Can you work these out from the model? Positions are in its coordinate system, mm. Face numbers are marked on the shaded views. A direction names the side the tool comes from. Coordinates: 2 decimals unless noted, no trailing zeros. Order: outer loops, then holes, each group sorted by start corner. A loop starts at its lowest first (then second) coordinate and runs counter-clockwise, first axis right, second up. Notation, with made-up numbers: M 59,65 L 95,65 A8 ccw 95,79 Z; hole C 33,-38 d2. An arc over 180 degrees is marked long. Answer as CSV lines item,"result". Start each with the question number.
1. I need wall thicknesses on line 1 along Z through (x, y) = (-30, 8.25); line 2 along Y through (x, z) = (-24, 19.5); line 3 along Y through (x, z) = (23, 33). Which ranges of each line are inside material? Lowest first, please. Write a range as from..to.
2. If we section it at A-A (x = 0): List the corners of the cut face in (y, z) for me, plus the area to 3 significant figures.
3. If we mould it in two halves opening along Y, with no side actions, what happens to the marked faces 6, 7 and 8? For each: released by +Y, released by -Y, zero draft, split by the parting line, or undercut.
4. Will these pins go through, and if not, where does the flat tip stop? pin 1 (3 mm diameter, centred on y = 23.5, z = 6.5, fed in from -X); pin 2 (3 mm diameter, centred on y = 25.5, z = 4.5, fed in from +X); pin 3 (2 mm diameter, centred on y = 45, z = 11.5, fed in from -X); pin 4 (8 mm diameter, centred on x = 36, z = 29, fed in from +Y).
5. If we section it at B-B (x = 31): List the corners of the cut face in (y, z) for me, plus the area to 3 significant figures.
6. On a 3-axis mill with a long thin cutter (end or side, diameter ignored), from which of +Z, -Z, +X, -X, +Y, -Y can I reach the whole of each face in a straight line? I mean the marked faces 1, 2, 3, 4 and 5. Say none if no direction works.
7. If we section it at C-C (z = 31.5): List the corners of the cut face in (x, y) for me.
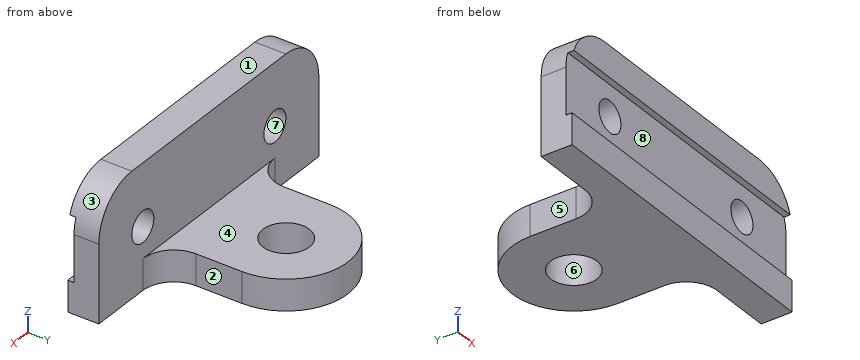
```python
from build123d import *
from OCP.BRepFilletAPI import BRepFilletAPI_MakeFillet

# Parameters (mm, degrees)
BASE_AND_EAR_PROFILE_SKETCH_W       = 100
BASE_AND_EAR_PROFILE_SKETCH_H       = 10
BASE_PLATE_DEPTH                    = 40
SKETCH1_3_R                         = 20
SKETCH1_3_R_2                       = 7.5
CLEVIS_EAR_DEPTH                    = 10
MOUNTING_HOLES_2X_REACH             = 80.262
MOUNTING_HOLES_SKETCH_R             = 5
MOUNTING_HOLES_2X_DIRECTION_2_DEPTH = 79.262379212
CORNER_AND_EAR_FILLETS_R1           = 10
CORNER_AND_EAR_FILLETS_R2           = 15
BOTTOM_GROOVE_DEPTH                 = 85.409715081
BOTTOM_GROOVE_DEPTH_BACK            = 85.409715081
BOTTOM_GROOVE_SKETCH_W              = 20
BOTTOM_GROOVE_SKETCH_H              = 2


with BuildPart() as part:
    # Base and Ear Profile Sketch → Base Plate (new body)
    with BuildSketch(Plane.XY):
        with Locations((0, 5)):
            Rectangle(BASE_AND_EAR_PROFILE_SKETCH_W, BASE_AND_EAR_PROFILE_SKETCH_H)
    extrude(amount=BASE_PLATE_DEPTH)

    # Sketch1_3 → Clevis Ear (add)
    # profile 1 of 2: a face of its own
    with BuildSketch(Plane.XY):
        with BuildLine():
            Line((-20, 35), (-20, 10))
            Line((-20, 10), (20, 10))
            Line((20, 10), (20, 35))
            ThreePointArc((20, 35), (0, 15), (-20, 35))
        make_face()
    # profile 2 of 2: a face of its own
    with BuildSketch(Plane.XY):
        with Locations((0, 35)):
            Circle(SKETCH1_3_R)
        with Locations((0, 35)):
            Circle(SKETCH1_3_R_2, mode=Mode.SUBTRACT)
    extrude(amount=CLEVIS_EAR_DEPTH)

    # Mounting Holes Sketch → Mounting Holes 2x (cut, up to next)
    with BuildSketch(Plane(origin=(0, 10, 0), x_dir=(1, 0, 0), z_dir=(0, 1, 0)), mode=Mode.PRIVATE) as mounting_holes_2x_sk1:
        with Locations(Location((30, -20, 0), (0, 0, 180))):
            Circle(MOUNTING_HOLES_SKETCH_R)
    mounting_holes_2x_tool1 = extrude(mounting_holes_2x_sk1.sketch, amount=-MOUNTING_HOLES_2X_REACH, mode=Mode.PRIVATE) & part.part
    # Mounting Holes Sketch → Mounting Holes 2x (cut, up to next)
    with BuildSketch(Plane(origin=(0, 10, 0), x_dir=(1, 0, 0), z_dir=(0, 1, 0)), mode=Mode.PRIVATE) as mounting_holes_2x_sk2:
        with Locations(Location((-30, -20, 0), (0, 0, 180))):
            Circle(MOUNTING_HOLES_SKETCH_R)
    mounting_holes_2x_tool2 = extrude(mounting_holes_2x_sk2.sketch, amount=-MOUNTING_HOLES_2X_REACH, mode=Mode.PRIVATE) & part.part
    add(mounting_holes_2x_tool1.solids().sort_by_distance((30, 10, 20))[0], mode=Mode.SUBTRACT)
    add(mounting_holes_2x_tool2.solids().sort_by_distance((-30, 10, 20))[0], mode=Mode.SUBTRACT)

    # Mounting Holes Sketch → Mounting Holes 2x direction 2 (cut)
    with BuildSketch(Plane(origin=(0, 10, 0), x_dir=(1, 0, 0), z_dir=(0, 1, 0))):
        with Locations(Location((30, -20, 0), (0, 0, 180))):
            Circle(MOUNTING_HOLES_SKETCH_R)
        with Locations(Location((-30, -20, 0), (0, 0, 180))):
            Circle(MOUNTING_HOLES_SKETCH_R)
    extrude(amount=MOUNTING_HOLES_2X_DIRECTION_2_DEPTH, mode=Mode.SUBTRACT)

    # Corner and Ear Fillets: one fillet with a radius per group of edges: ONE call of the kernel's fillet builder (fillet() takes one radius for all edges)
    corner_and_ear_fillets_edges_1 = [part.edges().sort_by_distance(p)[0] for p in [
        (20, 10, 5),
        (-20, 10, 5),
    ]]
    corner_and_ear_fillets_edges_2 = [part.edges().sort_by_distance(p)[0] for p in [
        (-50, 5, 40),
        (50, 5, 40),
    ]]
    corner_and_ear_fillets = BRepFilletAPI_MakeFillet(part.part.solid().wrapped)
    for e in corner_and_ear_fillets_edges_1:
        corner_and_ear_fillets.Add(CORNER_AND_EAR_FILLETS_R1, e.wrapped)
    for e in corner_and_ear_fillets_edges_2:
        corner_and_ear_fillets.Add(CORNER_AND_EAR_FILLETS_R2, e.wrapped)
    add(Compound.cast(corner_and_ear_fillets.Shape()), mode=Mode.REPLACE)

    # Bottom Groove Sketch → Bottom Groove (cut, two sides: drawn at the far end of the back side and taken through both)
    with BuildSketch(Plane(origin=(0, 0, 0), x_dir=(0, 0, -1), z_dir=(1, 0, 0)).offset(-BOTTOM_GROOVE_DEPTH_BACK)):
        with Locations((-20, 1)):
            Rectangle(BOTTOM_GROOVE_SKETCH_W, BOTTOM_GROOVE_SKETCH_H)
    extrude(amount=BOTTOM_GROOVE_DEPTH + BOTTOM_GROOVE_DEPTH_BACK, mode=Mode.SUBTRACT)


solid = part.part
```
Solved:
1,line 1,"0..15, 25..40"
1,line 2,"2..10"
1,line 3,"0..10"
2,outline,"M 0,0 L 27.5,0 L 27.5,10 L 10,10 L 10,40 L 0,40 L 0,30 L 2,30 L 2,10 L 0,10 Z; M 42.5,0 L 55,0 L 55,10 L 42.5,10 Z"
2,area,"660 mm²"
3,face 6,"undercut"
3,face 7,"zero draft"
3,face 8,"released by -Y"
4,pin 1,"x = -20"
4,pin 2,"x = 20"
4,pin 3,"through"
4,pin 4,"y = 10"
5,outline,"M 0,0 L 10,0 L 10,15.1 L 2,15.1 L 2,10 L 0,10 Z; M 0,30 L 2,30 L 2,24.9 L 10,24.9 L 10,40 L 0,40 Z"
5,area,"282 mm²"
6,face 1,"+Z, +X, -X, +Y, -Y"
6,face 2,"+Z, -Z, +X, +Y"
6,face 3,"+Z, +X, +Y, -Y"
6,face 4,"+Z, +X, -X, +Y"
6,face 5,"+Z, -Z, -X, +Y"
7,outline,"M -48.52,0 L 48.52,0 L 48.52,10 L -48.52,10 Z"
